The figure shows three views and two pictorial views of one solid part (mm, origin at its lowest corner). Answer the questions. Round coordinates to 2 decimals unless told otherwise and drop trailing zeros. Order: outer loops, then holes, each group sorted by start corner. A loop starts at its lowest first (then second) coordinate and runs counter-clockwise, first axis right, second up.
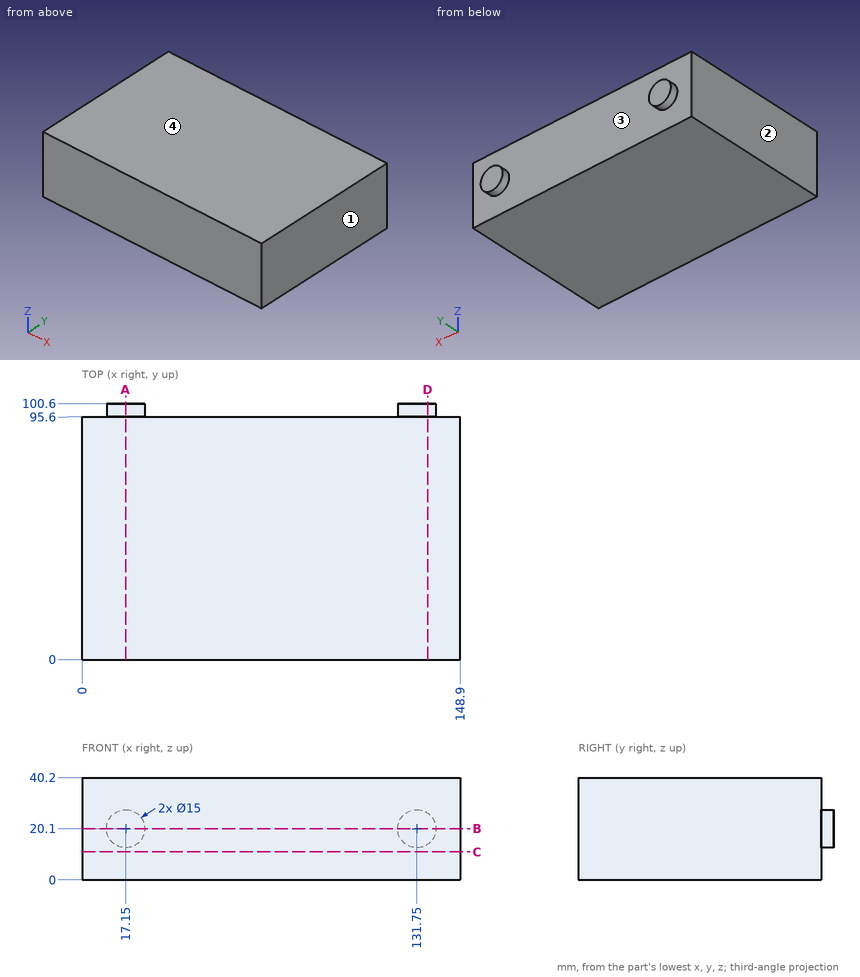
Item 1: Find the intervals of material crossed by line 1 along Y through (x, z) = (55, 27), in increasing order.
Item 2: For a pull along X with two mould halves and no side action, classify the marked faces 1, 2, 3 and 4 as released by +X, released by -X, zero draft, split by the parting line, or undercut.
Item 3: Find section B-B (z = 20.1). Write down the section's boundary in (x, y), plus the area to 3 significant figures.
Item 4: Find section A-A (x = 17.15). Write down the section's boundary in (y, z).
Item 5: Find section C-C (z = 11). Write down the section's boundary in (x, y).
Item 6: Given pin 1 (12 mm diameter, centred on x = 87.5, z = 30, fed in from +Y); pin 2 (2 mm diameter, centred on x = 21, z = 5, fed in from -Y), each flat-ended and moving along its own axis, determine where each tip first touches the part or whether it passes through.
Item 7: Find section D-D (x = 136). Write down the section's boundary in (y, z).
Model answer:
1. line 1: y = 0 to 95.6
2. face 1: released by +X
2. face 2: released by -X
2. face 3: undercut
2. face 4: zero draft
3. outline: (0, 0) - (148.9, 0) - (148.9, 95.6) - (139.25, 95.6) - (139.25, 100.6) - (124.25, 100.6) - (124.25, 95.6) - (24.65, 95.6) - (24.65, 100.6) - (9.65, 100.6) - (9.65, 95.6) - (0, 95.6) - close
3. area: 14,400 mm2
4. outline: (0, 0) - (95.6, 0) - (95.6, 12.6) - (100.6, 12.6) - (100.6, 27.6) - (95.6, 27.6) - (95.6, 40.2) - (0, 40.2) - close
5. outline: (0, 0) - (148.9, 0) - (148.9, 95.6) - (0, 95.6) - close
6. pin 1: stops at y = 95.6
6. pin 2: stops at y = 0
7. outline: (0, 0) - (95.6, 0) - (95.6, 13.92) - (100.6, 13.92) - (100.6, 26.28) - (95.6, 26.28) - (95.6, 40.2) - (0, 40.2) - close
